The model under review builds one solid part; all positions refer to its coordinate system, in mm. A direction names the side the tool comes from. Coordinates: 2 decimals unless noted, no trailing zeros. Order: outer loops, then holes, each group sorted by start corner. A loop starts at its lowest first (then second) coordinate and runs counter-clockwise, first axis right, second up. Notation, with made-up numbers: M 18,37.5 L 75,37.5 A5 cw 75,42.5 Z; hole C 68,-23.5 d10. An arc over 180 degrees is marked long. Answer in a Markdown table with one row per item.
from build123d import *

# Parameters (mm, degrees)
CHAMFER1_SIZE           = 1
FILLET1_R               = 1
SKETCH2_OUTSIDE_W       = 78.154
SKETCH2_OUTSIDE_H       = 78.154
SKETCH2_OUTSIDE_W_2     = 80
SKETCH2_OUTSIDE_H_2     = 45
CUT_EXTRUDE1_DEPTH      = 6
CUT_EXTRUDE2_DEPTH      = 116.027170703
CUT_EXTRUDE2_DEPTH_BACK = 116.027170703
SKETCH3_R               = 3.15
CUT_EXTRUDE3_DEPTH      = 116.027170703
CUT_EXTRUDE3_DEPTH_BACK = 116.027170703
SKETCH4_R               = 3.15


with BuildPart() as part:
    # Sketch1 → Revolve1 (revolve)
    with BuildSketch(Plane.XY, mode=Mode.PRIVATE) as revolve1_sk:
        Polygon((0, 0), (25, 0), (25, 6), (20, 6), (20, 65), (15, 65), (15, 110), (0, 110), align=None)
    revolve(revolve1_sk.sketch.rotate(Axis((0, 0, 0), (0, -1, 0)), 90), axis=Axis((0, 0, 0), (0, -1, 0)))

    # Chamfer1
    chamfer1_edges = [part.edges().sort_by_distance(p)[0] for p in [
        (0, 110, -15),
        (0, 65, -20),
        (0, 6, -25),
        (0, 0, -25),
    ]]
    chamfer(chamfer1_edges, length=CHAMFER1_SIZE)

    # Fillet1
    fillet1_edges = [part.edges().sort_by_distance(p)[0] for p in [
        (0, 65, -15),
        (0, 6, -20),
    ]]
    fillet(fillet1_edges, radius=FILLET1_R)

    # Sketch2 outside → Cut-Extrude1 (cut)
    with BuildSketch(Plane(origin=(0, 0, 0), x_dir=(1, 0, 0), z_dir=(0, 1, 0))):
        Rectangle(SKETCH2_OUTSIDE_W, SKETCH2_OUTSIDE_H)
        Rectangle(SKETCH2_OUTSIDE_W_2, SKETCH2_OUTSIDE_H_2, mode=Mode.SUBTRACT)
    extrude(amount=CUT_EXTRUDE1_DEPTH, mode=Mode.SUBTRACT)

    # Sketch3 → Cut-Extrude2 (cut, two sides: drawn at the far end of the back side and taken through both)
    with BuildSketch(Plane.XY.offset(-CUT_EXTRUDE2_DEPTH_BACK)):
        with Locations(Location((0, 103, 0), (0, 0, 269.99999995))):
            Circle(SKETCH3_R)
    extrude(amount=CUT_EXTRUDE2_DEPTH + CUT_EXTRUDE2_DEPTH_BACK, mode=Mode.SUBTRACT)

    # Sketch4 → Cut-Extrude3 (cut, two sides: drawn at the far end of the back side and taken through both)
    with BuildSketch(Plane(origin=(0, 0, 0), x_dir=(0, 0, -1), z_dir=(1, 0, 0)).offset(-CUT_EXTRUDE3_DEPTH_BACK)):
        with Locations((0, 95)):
            Circle(SKETCH4_R)
    extrude(amount=CUT_EXTRUDE3_DEPTH + CUT_EXTRUDE3_DEPTH_BACK, mode=Mode.SUBTRACT)


solid = part.part
(1) Take a section at D-D (y = 103). Write out the cut boundary in (x, z).
Report:
| item | result |
|---|---|
| outline | M -3.15,-14.67 L -3.15,14.67 A15 ccw Z; M 3.15,-14.67 A15 ccw 3.15,14.67 Z |
(2) Take a section at C-C (y = 74). Write out the cut boundary in (x, z).
Report:
| item | result |
|---|---|
| outline | C 0,0 d30 |
(3) To check wall thickness, follow line 1 (Y direction, x = -8, z = 0); line 2 (Z direction, x = 6.5, y = 95); line 3 (X direction, y = 103, z = -1). State the ranges of each line that lie inside material, in increasing order. Write a range as [from, to].
Report:
| item | result |
|---|---|
| line 1 | [0, 91.85], [98.15, 110] |
| line 2 | [-13.52, -3.15], [3.15, 13.52] |
| line 3 | [-14.97, -3.15], [3.15, 14.97] |
(4) The part is to be moulded in two halves that separate along Y. For faces 3 (the flat face through (7, 6, -20)), 4 (the cylindrical face through (-0.21, 98.123, 0.41)), 5 (the flat face through (0, 0, 0)), say which applies: +Y half, -Y half, draft (parallel to the pull), parting line (faces both ways), or undercut.
Report:
| item | result |
|---|---|
| face 3 | +Y half |
| face 4 | undercut |
| face 5 | -Y half |
(5) Take a section at A-A (x = 0). Write out the cut boundary in (y, z).
Report:
| item | result |
|---|---|
| outline | M 0,-22.5 L 6,-22.5 L 6,-21 A1 cw 7,-20 L 64,-20 L 65,-19 L 65,-16 A1 cw 66,-15 L 99.85,-15 L 99.85,15 L 66,15 A1 cw 65,16 L 65,19 L 64,20 L 7,20 A1 cw 6,21 L 6,22.5 L 0,22.5 Z; M 106.15,-15 L 109,-15 L 110,-14 L 110,14 L 109,15 L 106.15,15 Z; hole C 95,0 d6.3 |
(6) Machinability: for faces 1 (the conical face through (24.17, 0.174, -0.411)), 2 (the cylindrical face through (-0.88, 35.9, -19.98)), which of the approach directions +Z, -Z, +X, -X, +Y, -Y give a long, thin tool a straight path to every point of the face, cutting with its end or side? Answer none if there is none.
Report:
| item | result |
|---|---|
| face 1 | +X, -Y |
| face 2 | +Y |
(7) Take a section at B-B (z = 0). State how many separate pieces and enclosed holes the cut face has, then the cut area to 3 significant figures.
Report:
| item | result |
|---|---|
| separate pieces | 2 |
| enclosed holes | 1 |
| area | 3,790 mm^2 |
(8) Insertion check: P1, Ø12, axis at x = -19.5, y = 85.5, coming from the +Z side; P2, Ø6, axis at x = -13, y = 22.5, coming from the -Z side; P3, Ø12, axis at x = 16, y = 17.5, coming from the +Z side. Each pin has a flat end and moves straight along its axis. Give the tip position at first contact, or say it passes through.
Report:
| item | result |
|---|---|
| P1 | z = 6.54 |
| P2 | z = -17.32 |
| P3 | z = 17.32 |
